from build123d import *

# Parameters (mm, degrees)
BASE_BLOCK_DEPTH        = 20
STEP_PAD_1_DEPTH        = 5
STEP_START              = -5
STEP_PAD_2_DEPTH        = 5
ROUND_BOSS_SKETCH_R     = 20
ROUND_BOSS_DEPTH        = 20
RISER_BLOCK_1_DEPTH     = 20
SIDE_PAD_1_SKETCH_W     = 40
SIDE_PAD_1_SKETCH_H     = 10
SIDE_PAD_1_DEPTH        = 5
RISER_BLOCK_2_SKETCH_W  = 40
RISER_BLOCK_2_SKETCH_H  = 10
RISER_BLOCK_2_DEPTH     = 20
SIDE_PAD_2_SKETCH_W     = 40
SIDE_PAD_2_SKETCH_H     = 10
SIDE_PAD_2_DEPTH        = 5
RISER_BLOCK_3_SKETCH_W  = 40
RISER_BLOCK_3_SKETCH_H  = 10
RISER_BLOCK_3_DEPTH     = 20
BORE_20_SKETCH_R        = 10
BORE_20_DEPTH           = 76
CORNER_SLOT_1_SKETCH_W  = 5
CORNER_SLOT_1_SKETCH_H  = 5
CORNER_SLOT_1_5X5_DEPTH = 25
CORNER_SLOT_2_SKETCH_W  = 5
CORNER_SLOT_2_SKETCH_H  = 5
CORNER_SLOT_2_5X5_DEPTH = 25
HOLE_1_DEPTH            = 16
HOLE_1_DEPTH_BACK       = 53
HOLE_1_SKETCH_R         = 5
HOLE_2_SKETCH_R         = 5
HOLE_2_DEPTH            = 122
TOP_BLOCK_SKETCH_W      = 5
TOP_BLOCK_SKETCH_H      = 10
TOP_BLOCK_45_DEPTH      = 25


with BuildPart() as part:
    # Base Profile Sketch → Base Block (new body)
    with BuildSketch(Plane(origin=(0, 0, 0), x_dir=(1, 0, 0), z_dir=(0, 1, 0))):
        with BuildLine():
            Line((8.306767896, 1.392410292), (8.306767896, 31.392410292))
            Line((8.306767896, 31.392410292), (-51.693232104, 31.392410292))
            ThreePointArc((-51.693232104, 31.392410292), (-81.693232104, 1.392410292), (-51.693232104, -28.607589708))
            Line((-51.693232104, -28.607589708), (8.306767896, -28.607589708))
            Line((8.306767896, -28.607589708), (8.306767896, 1.392410292))
        make_face()
    extrude(amount=BASE_BLOCK_DEPTH)

    # Step Pad 1 Sketch → Step Pad 1 (add)
    with BuildSketch(Plane(origin=(0, 20, 0), x_dir=(1, 0, 0), z_dir=(0, 1, 0))):
        with BuildLine():
            ThreePointArc((-31.693232104, 1.392410292), (-37.55109648, 15.534545916), (-51.693232104, 21.392410292))
            ThreePointArc((-51.693232104, 21.392410292), (-71.693232104, 1.392410292), (-51.693232104, -18.607589708))
            ThreePointArc((-51.693232104, -18.607589708), (-37.55109648, -12.749725331), (-31.693232104, 1.392410292))
        make_face()
    extrude(amount=STEP_PAD_1_DEPTH)

    # Step Pad 2 Sketch → Step Pad 2 (add)
    with BuildSketch(Plane(origin=(0, 25, 0), x_dir=(1, 0, 0), z_dir=(0, 1, 0)).offset(STEP_START)):
        with BuildLine():
            Line((-51.693232104, 21.392410292), (8.306767896, 21.392410292))
            Line((8.306767896, 21.392410292), (8.306767896, -18.607589708))
            Line((8.306767896, -18.607589708), (-51.693232104, -18.607589708))
            ThreePointArc((-51.693232104, -18.607589708), (-71.693232104, 1.392410292), (-51.693232104, 21.392410292))
        make_face()
    extrude(amount=STEP_PAD_2_DEPTH)

    # Round Boss Sketch → Round Boss (add)
    with BuildSketch(Plane(origin=(0, 25, 0), x_dir=(1, 0, 0), z_dir=(0, 1, 0))):
        with Locations(Location((-51.693232104, 1.392410292, 0), (0, 0, 270))):
            Circle(ROUND_BOSS_SKETCH_R)
    extrude(amount=ROUND_BOSS_DEPTH)

    # Riser Block 1 Sketch → Riser Block 1 (add)
    with BuildSketch(Plane(origin=(0, 25, 0), x_dir=(1, 0, 0), z_dir=(0, 1, 0))):
        with BuildLine():
            Line((8.306767896, 21.392410292), (-51.693232104, 21.392410292))
            ThreePointArc((-51.693232104, 21.392410292), (-31.693232104, 1.392410292), (-51.693232104, -18.607589708))
            Line((-51.693232104, -18.607589708), (8.306767896, -18.607589708))
            Line((8.306767896, -18.607589708), (8.306767896, 21.392410292))
        make_face()
    extrude(amount=RISER_BLOCK_1_DEPTH)

    # Side Pad 1 Sketch → Side Pad 1 (add)
    with BuildSketch(Plane(origin=(0, 20, 0), x_dir=(1, 0, 0), z_dir=(0, 1, 0))):
        with Locations((-11.693232104, 26.392410292)):
            Rectangle(SIDE_PAD_1_SKETCH_W, SIDE_PAD_1_SKETCH_H)
    extrude(amount=SIDE_PAD_1_DEPTH)

    # Riser Block 2 Sketch → Riser Block 2 (add)
    with BuildSketch(Plane(origin=(0, 25, 0), x_dir=(1, 0, 0), z_dir=(0, 1, 0))):
        with Locations((-11.693232104, 26.392410292)):
            Rectangle(RISER_BLOCK_2_SKETCH_W, RISER_BLOCK_2_SKETCH_H)
    extrude(amount=RISER_BLOCK_2_DEPTH)

    # Side Pad 2 Sketch → Side Pad 2 (add)
    with BuildSketch(Plane(origin=(0, 20, 0), x_dir=(1, 0, 0), z_dir=(0, 1, 0))):
        with Locations((-11.693232104, -23.607589708)):
            Rectangle(SIDE_PAD_2_SKETCH_W, SIDE_PAD_2_SKETCH_H)
    extrude(amount=SIDE_PAD_2_DEPTH)

    # Riser Block 3 Sketch → Riser Block 3 (add)
    with BuildSketch(Plane(origin=(0, 25, 0), x_dir=(1, 0, 0), z_dir=(0, 1, 0))):
        with Locations((-11.693232104, -23.607589708)):
            Rectangle(RISER_BLOCK_3_SKETCH_W, RISER_BLOCK_3_SKETCH_H)
    extrude(amount=RISER_BLOCK_3_DEPTH)

    # Bore Ø20 Sketch → Bore Ø20 (cut)
    with BuildSketch(Plane(origin=(0, 45, 0), x_dir=(1, 0, 0), z_dir=(0, 1, 0))):
        with Locations(Location((-51.693232104, 1.392410292, 0), (0, 0, 270))):
            Circle(BORE_20_SKETCH_R)
    extrude(amount=-BORE_20_DEPTH, mode=Mode.SUBTRACT)

    # Corner Slot 1 Sketch → Corner Slot 1 5x5 (cut)
    with BuildSketch(Plane(origin=(0, 45, 0), x_dir=(1, 0, 0), z_dir=(0, 1, 0))):
        with Locations((5.806767896, 28.892410292)):
            Rectangle(CORNER_SLOT_1_SKETCH_W, CORNER_SLOT_1_SKETCH_H)
    extrude(amount=-CORNER_SLOT_1_5X5_DEPTH, mode=Mode.SUBTRACT)

    # Corner Slot 2 Sketch → Corner Slot 2 5x5 (cut)
    with BuildSketch(Plane(origin=(0, 45, 0), x_dir=(1, 0, 0), z_dir=(0, 1, 0))):
        with Locations((5.806767896, -26.107589708)):
            Rectangle(CORNER_SLOT_2_SKETCH_W, CORNER_SLOT_2_SKETCH_H)
    extrude(amount=-CORNER_SLOT_2_5X5_DEPTH, mode=Mode.SUBTRACT)

    # Hole 1 Sketch → Hole 1 (cut, two sides: drawn at the far end of the back side and taken through both)
    with BuildSketch(Plane(origin=(0, 45, 0), x_dir=(1, 0, 0), z_dir=(0, 1, 0)).offset(-HOLE_1_DEPTH_BACK)):
        with Locations(Location((-1.693232104, -13.607589708, 0), (0, 0, 270))):
            Circle(HOLE_1_SKETCH_R)
    extrude(amount=HOLE_1_DEPTH + HOLE_1_DEPTH_BACK, mode=Mode.SUBTRACT)

    # Hole 2 Sketch → Hole 2 (cut)
    with BuildSketch(Plane(origin=(0, 45, 0), x_dir=(1, 0, 0), z_dir=(0, 1, 0))):
        with Locations(Location((-1.693232104, 16.392410292, 0), (0, 0, 270))):
            Circle(HOLE_2_SKETCH_R)
    extrude(amount=-HOLE_2_DEPTH, mode=Mode.SUBTRACT)

    # Top Block Sketch → Top Block 45 (add)
    with BuildSketch(Plane(origin=(0, 20, 0), x_dir=(1, 0, 0), z_dir=(0, 1, 0))):
        with Locations((-34.193232104, 26.392410292)):
            Rectangle(TOP_BLOCK_SKETCH_W, TOP_BLOCK_SKETCH_H)
        with Locations((-34.193232104, -23.607589708)):
            Rectangle(TOP_BLOCK_SKETCH_W, TOP_BLOCK_SKETCH_H)
    extrude(amount=TOP_BLOCK_45_DEPTH)


solid = part.part
Design review of the part built by this model. Coordinates are the model's own, in mm. A direction names the side the tool comes from. Coordinates: 2 decimals unless noted, no trailing zeros. Order: outer loops, then holes, each group sorted by start corner. A loop starts at its lowest first (then second) coordinate and runs counter-clockwise, first axis right, second up. Notation, with made-up numbers: M 20,21 L 77,21 A7 cw 77,32 Z; hole C 52,73.5 d10. An arc over 180 degrees is marked long. Use a Markdown table: item, result.
(1) Add section A-A (z = -3). Give the boundary of the cut face in (x, y).
Worked answers:
| item | result |
|---|---|
| outline | M -81.65,0 L -61.56,0 L -61.56,45 L -71.63,45 L -71.63,20 L -81.65,20 Z; M -41.82,0 L 8.31,0 L 8.31,45 L -41.82,45 Z |
(2) Add section B-B (x = -54). Give the boundary of the cut face in (y, z).
Worked answers:
| item | result |
|---|---|
| outline | M 0,-31.3 L 20,-31.3 L 20,-21.26 L 45,-21.26 L 45,-11.12 L 0,-11.12 Z; M 0,8.34 L 45,8.34 L 45,18.47 L 20,18.47 L 20,28.52 L 0,28.52 Z |
(3) For P1, Ø16.5, axis at x = -46, y = 29.5, coming from the -Z side; P2, Ø16, axis at x = -51.69, z = -1.39, coming from the +Y side; P3, Ø3, axis at y = 29, z = 23.5, coming from the -X side; P4, Ø12, axis at x = -72, y = 33, coming from the -Z side, all flat-tipped, find the tip position at first contact; note any pin that passes through.
Worked answers:
| item | result |
|---|---|
| P1 | stops at z = -21.39 |
| P2 | passes through |
| P3 | stops at x = -36.69 |
| P4 | stops at z = -15.37 |
(4) For faces 1 (the flat face through (3.307, 33, -29)), 2 (the flat face through (-44, 32, -21.392)), 3 (the flat face through (-36.693, 32, 24)), 4 (the flat face through (-75, 20, -2)), 5 (the flat face through (6, 20, 26)), list the 3-axis set-ups (+Z, -Z, +X, -X, +Y, -Y) from which the entire face can be reached by the end or side of a thin tool; tool diameter is ignored.
Worked answers:
| item | result |
|---|---|
| face 1 | -Z, +X, +Y |
| face 2 | -Z, -X, +Y |
| face 3 | +Z, -X, +Y |
| face 4 | -X, +Y |
| face 5 | +Z, +X, +Y |
(5) Wall thickness on probe 1 along Z at (x, y) = (-2, 20); probe 2 along X at (y, z) = (40.5, -24); probe 3 along X at (y, z) = (39, -17.5): over which ranges is each line inside the solid? List them lowest first.
Worked answers:
| item | result |
|---|---|
| probe 1 | z = -31.39 to -21.38, -11.4 to 8.62, 18.6 to 28.61 |
| probe 2 | x = -36.69 to 8.31 |
| probe 3 | x = -63.55 to -6.57, 3.18 to 8.31 |
(6) Add section C-C (y = 16). Give the boundary of the cut face in (x, z).
Worked answers:
| item | result |
|---|---|
| outline | M -51.69,-31.39 L 8.31,-31.39 L 8.31,28.61 L -51.69,28.61 A30 ccw Z; hole C -51.69,-1.39 d20; hole C -1.69,-16.39 d10; hole C -1.69,13.61 d10 |
(7) Draft analysis for pull direction Z (two halves, no side actions). For faces 6 (the flat face through (-36.693, 32, -26)), 7 (the flat face through (-44, 32, 18.608)), 8 (the cylindrical face through (-0.191, 22.185, 18.377)), state which applies: released by +Z, released by -Z, zero draft, split by the parting line, or undercut.
Worked answers:
| item | result |
|---|---|
| face 6 | zero draft |
| face 7 | released by +Z |
| face 8 | undercut |
(8) Add section D-D (z = -16.5). Give the boundary of the cut face in (x, y).
Worked answers:
| item | result |
|---|---|
| outline | M -77.61,0 L -6.69,0 L -6.69,45 L -64.8,45 L -64.8,20 L -77.61,20 Z; M 3.31,0 L 8.31,0 L 8.31,45 L 3.31,45 Z |
